Verification items for this drawing (mm, ordinates from the low corner). A direction names the side the tool comes from. Coordinates: 2 decimals unless noted, no trailing zeros. Loops run counter-clockwise (first coordinate to the right, second up) from the corner with the lowest first, then second, coordinate; pieces in that order, holes last. Notation, with made-up numbers: M -26,-1 L -8,-1 A28 ccw -8,17 Z; hole C -30.5,80.5 d5. An arc over 180 degrees is marked long. Use CSV: the item, a comma, the result in double quotes.
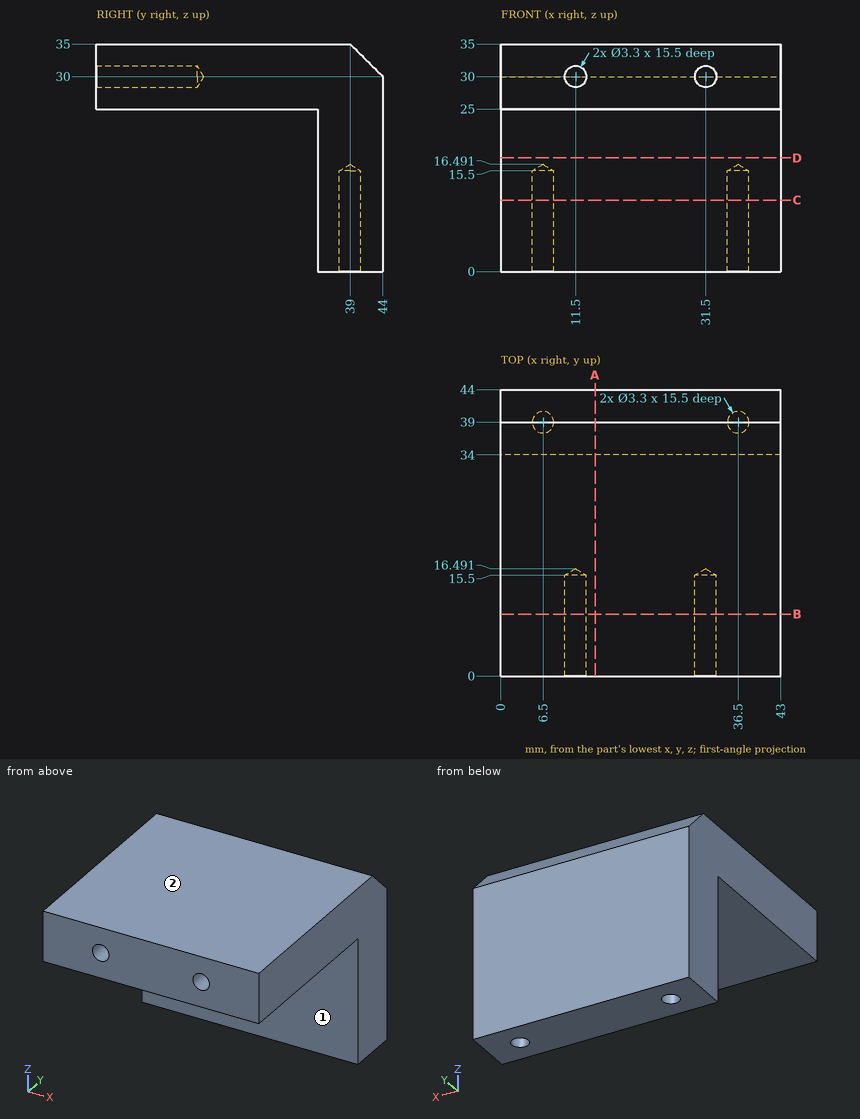
1. Set-up check for the marked faces 1 and 2: record each of +Z, -Z, +X, -X, +Y, -Y from which the full face is reachable in a straight line by a thin tool's end or side.
The answers:
face 1,"-Z, +X, -X, -Y"
face 2,"+Z, +X, -X, +Y, -Y"
2. Section check A-A, the plane x = 14.5. Record the cut outline in (y, z).
The answers:
outline,"M 0,25 L 34,25 L 34,0 L 44,0 L 44,30 L 39,35 L 0,35 Z"
3. Section check C-C, the plane z = 11. Record the cut outline in (x, y), plus the area to 3 significant figures.
The answers:
outline,"M 0,34 L 43,34 L 43,44 L 0,44 Z; hole C 6.5,39 d3.3; hole C 36.5,39 d3.3"
area,"413 mm^2"
4. Gauge pin test, flat ends, axial feed: P1, Ø4.5, axis at x = 11.5, z = 30, coming from the -Y side; P2, Ø10, axis at x = 26.5, y = 22, coming from the -Z side; P3, Ø7.5, axis at x = 21, z = 17, coming from the -Y side. Record the tip position at first contact, or that the pin passes through.
The answers:
P1,"y = 0"
P2,"z = 25"
P3,"y = 34"
5. Thickness scan on line 1 (X direction, y = 39, z = 11); line 2 (X direction, y = 5.25, z = 30); line 3 (Z direction, x = 31.5, y = 9.5). Record the ranges inside material, lowest first. Write a range as [from, to].
The answers:
line 1,"[0, 4.85], [8.15, 34.85], [38.15, 43]"
line 2,"[0, 9.85], [13.15, 29.85], [33.15, 43]"
line 3,"[25, 28.35], [31.65, 35]"
6. Section check B-B, the plane y = 9.5. Record the cut outline in (x, z).
The answers:
outline,"M 0,25 L 43,25 L 43,35 L 0,35 Z; hole C 11.5,30 d3.3; hole C 31.5,30 d3.3"
7. Section check D-D, the plane z = 17.5. Record the cut outline in (x, y).
The answers:
outline,"M 0,34 L 43,34 L 43,44 L 0,44 Z"
